For this review, use the dimensioned drawing (mm, ordinates from the lowest corner) and the shaded views. A direction names the side the tool comes from. Round coordinates to 2 decimals unless told otherwise and drop trailing zeros. Order: outer loops, then holes, each group sorted by start corner. A loop starts at its lowest first (then second) coordinate and runs counter-clockwise, first axis right, second up. Notation, with made-up numbers: M 54,-33 L 62,-33 A31 ccw 62,1 Z; hole C -20,-26.5 d9. An arc over 180 degrees is marked long. Answer as CSV lines item,"result". Start each with the question number.
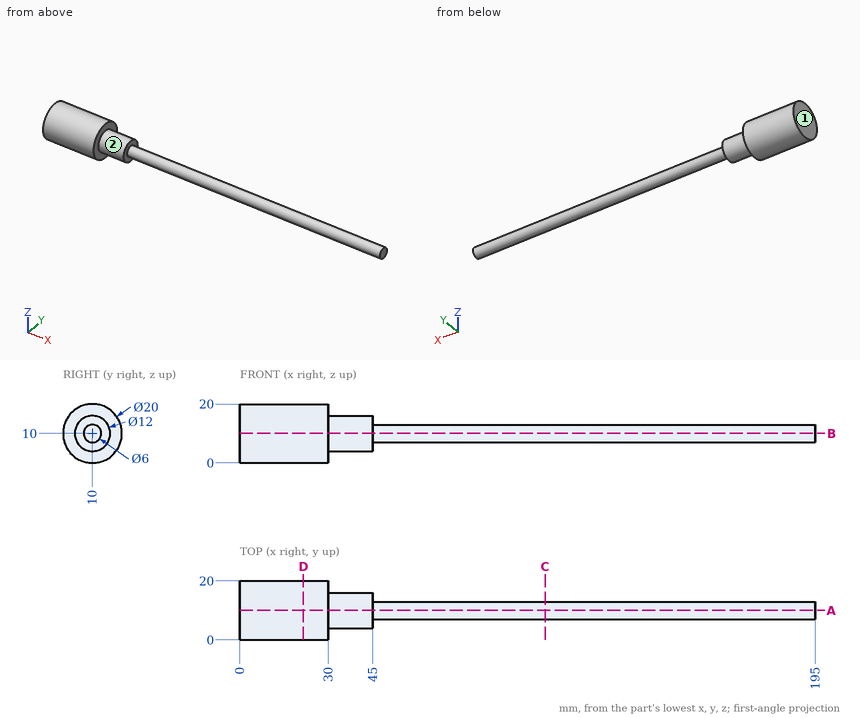
Item 1: Consider section D-D (x = 21.5). State the section outline as (y, z) points, and give its area (3 significant figures).
Item 2: Wall thickness on probe 1 along X at (y, z) = (6.25, 18); probe 2 along Z at (x, y) = (43.5, 9.5); probe 3 along X at (y, z) = (8.25, 14.75): over which ranges is each line inside the solid? List them lowest first. Write a range as [from, to].
Item 3: Consider section A-A (y = 10). State the section outline as (x, z) points.
Item 4: Tool access review of the marked faces 1 and 2: name each direction out of +Z, -Z, +X, -X, +Y, -Y from which nothing blocks a thin tool from reaching the whole face with its end or side.
Item 5: For pin 1 (3 mm diameter, centred on y = 4, z = 16, fed in from +X), flat-tipped, find the tip position at first contact; note if it passes through.
Item 6: Consider section C-C (x = 103.5). State the section outline as (y, z) points.
Reported:
1,outline,"C 10,10 d20"
1,area,"314 mm²"
2,probe 1,"x = [0, 30]"
2,probe 2,"z = [4.02, 15.98]"
2,probe 3,"x = [0, 45]"
3,outline,"M 0,0 L 30,0 L 30,4 L 45,4 L 45,7 L 195,7 L 195,13 L 45,13 L 45,16 L 30,16 L 30,20 L 0,20 Z"
4,face 1,"+Z, -Z, -X, +Y, -Y"
4,face 2,"+X"
5,pin 1,"stops at x = 30"
6,outline,"C 10,10 d6"
